The listing builds one solid part. Answer for the finished solid, in the listing's coordinates (mm). A direction names the side the tool comes from. Coordinates: 2 decimals unless noted, no trailing zeros. Order: outer loops, then holes, each group sorted by start corner. A loop starts at its lowest first (then second) coordinate and runs counter-clockwise, first axis right, second up.
```python
from build123d import *
from build123d.topology import SkipClean

# Parameters (mm, degrees)
SKETCH2_R           = 24
BOSS_EXTRUDE1_DEPTH = 47
SKETCH3_R           = 26
BOSS_EXTRUDE2_DEPTH = 14
SKETCH5_R           = 16
BOSS_EXTRUDE3_DEPTH = 46
BOSS_EXTRUDE4_START = 28
BOSS_EXTRUDE4_DEPTH = 18
SKETCH8_R           = 20
CUT_EXTRUDE1_DEPTH  = 5
SKETCH12_R          = 12.5
CUT_EXTRUDE3_DEPTH  = 34
CUT_EXTRUDE4_START  = -25
SKETCH13_R          = 12.5
CUT_EXTRUDE4_DEPTH  = 25
SKETCH11_R          = 17.5
CUT_EXTRUDE2_DEPTH  = 39
SKETCH16_W          = 29
SKETCH16_H          = 2.5
SKETCH17_W          = 2.5
SKETCH17_H          = 11.435558067


with BuildPart() as part:
    # Sketch1 → Revolve1 (revolve)
    with BuildSketch(Plane.XY):
        with BuildLine():
            Line((-29, 0), (29, 0))
            ThreePointArc((29, 0), (0, 29), (-29, 0))
        make_face()
    revolve(axis=Axis((-1000, 0, 0), (1, 0, 0)))

    # Sketch2 → Boss-Extrude1 (add)
    with BuildSketch(Plane(origin=(0, 0, 0), x_dir=(1, 0, 0), z_dir=(0, 1, 0))):
        with Locations(Location((0, 0, 0), (0, 0, 90))):
            Circle(SKETCH2_R)
    extrude(amount=BOSS_EXTRUDE1_DEPTH)

    # Sketch3 → Boss-Extrude2 (add)
    with BuildSketch(Plane(origin=(0, 47, 0), x_dir=(1, 0, 0), z_dir=(0, 1, 0))):
        with Locations(Location((0, 0, 0), (0, 0, 270))):
            Circle(SKETCH3_R)
    extrude(amount=-BOSS_EXTRUDE2_DEPTH)

    # Sketch5 → Boss-Extrude3 (add)
    with BuildSketch(Plane.XY):
        with Locations(Location((0, 0, 0), (0, 0, 180))):
            Circle(SKETCH5_R)
    boss_extrude3 = extrude(amount=BOSS_EXTRUDE3_DEPTH)

    # Sketch4 → Boss-Extrude4 (add)
    with BuildSketch(Plane.XY.offset(BOSS_EXTRUDE4_START)):
        Polygon((20.784609691, 12), (0, 24), (-20.784609691, 12), (-20.784609691, -12), (0, -24), (20.784609691, -12), align=None)
    boss_extrude4 = extrude(amount=BOSS_EXTRUDE4_DEPTH)

    # Sketch8 → Cut-Extrude1 (cut)
    with BuildSketch(Plane(origin=(0, 47, 0), x_dir=(1, 0, 0), z_dir=(0, 1, 0))):
        with Locations(Location((0, 0, 0), (0, 0, 270))):
            Circle(SKETCH8_R)
    extrude(amount=-CUT_EXTRUDE1_DEPTH, mode=Mode.SUBTRACT)

    # Sketch12 → Cut-Extrude3 (cut)
    with BuildSketch(Plane.XY.offset(46)):
        Circle(SKETCH12_R)
    extrude(amount=-CUT_EXTRUDE3_DEPTH, mode=Mode.SUBTRACT)

    # Mirror1: Boss-Extrude3, Boss-Extrude4 across plane
    add(boss_extrude3.mirror(Plane.XY))
    add(boss_extrude4.mirror(Plane.XY))

    # Sketch13 → Cut-Extrude4 (cut)
    with BuildSketch(Plane(origin=(0, 0, -46), x_dir=(-1, 0, 0), z_dir=(0, 0, -1)).offset(CUT_EXTRUDE4_START)):
        with Locations(Location((0, 0, 0), (0, 0, 180))):
            Circle(SKETCH13_R)
    extrude(amount=CUT_EXTRUDE4_DEPTH, mode=Mode.SUBTRACT)

    # Sketch11 → Cut-Extrude2 (cut)
    with BuildSketch(Plane(origin=(0, 42, 0), x_dir=(1, 0, 0), z_dir=(0, 1, 0))):
        with Locations(Location((0, 0, 0), (0, 0, 270))):
            Circle(SKETCH11_R)
    extrude(amount=-CUT_EXTRUDE2_DEPTH, mode=Mode.SUBTRACT)

    # Sketch15 → Cut-Revolve1 (revolve, cut)
    with BuildSketch(Plane(origin=(0, 0, 0), x_dir=(0, 0, -1), z_dir=(1, 0, 0))):
        Polygon((-6.5, 3), (0, -3.5), (0, 11), (-6.5, 11), align=None)
    revolve(axis=Axis((0, -1000, 0), (0, 1, 0)), mode=Mode.SUBTRACT)

    # Sketch16 → Cut-Revolve2 (revolve, cut)
    with BuildSketch(Plane(origin=(0, 0, 0), x_dir=(0, 0, -1), z_dir=(1, 0, 0)), mode=Mode.PRIVATE) as cut_revolve2_sk:
        with Locations((12, -6.25)):
            Rectangle(SKETCH16_W, SKETCH16_H)
    revolve(cut_revolve2_sk.sketch.rotate(Axis((0, -5, 4.897022233), (0, 0, -1)), 270), axis=Axis((0, -5, 4.897022233), (0, 0, -1)), mode=Mode.SUBTRACT)

    # Sketch17 → Cut-Revolve3 (revolve, cut)
    with SkipClean():  # the faces are left unmerged after this step: merging them gives an invalid solid
        with BuildSketch(Plane(origin=(0, 0, 0), x_dir=(0, 0, -1), z_dir=(1, 0, 0))):
            with Locations((-1.25, 0.717779034)):
                Rectangle(SKETCH17_W, SKETCH17_H)
        revolve(axis=Axis((0, -5, 0), (0, 1, 0)), mode=Mode.SUBTRACT)


solid = part.part
```
(1) The mould has two halves that part along X. Classify faces 1 (the face through (20.785, 0, -37)), 2 (the face through (-1.6, 16.1, 28)), 3 (the face through (-1.639, -0.806, -2.138)): released by +X, released by -X, zero draft, split by the parting line, or undercut.
(2) Find section B-B (y = 10). Write down the section's boundary in (x, z).
(3) Find section C-C (z = -15). Write down the section's boundary in (x, y) (3 decimals).
(4) Each of these flat-tipped pins is pushed along its axis until it touches: pin 1 Ø20 at (y, z) = (4, 36) entering from -X; pin 2 Ø12.5 at (x, y) = (-0.5, 1.5) entering from +Z; pin 3 Ø12 at (y, z) = (-5, 5.5) entering from +X. Where does it stop, or does it pass through?
(5) Consider line 1 (X direction, y = 21, z = 0); line 2 (Y direction, x = 0, z = -27); line 3 (Z direction, x = 17.5, y = 1). Determine where each line is inside the solid, lowest interval first.
(6) Find section D-D (z = 22). Write down the section's boundary in (x, y).
(7) Find section A-A (z = -36.5). Write down the section's boundary in (x, y), and give its area (3 significant figures).
(8) For faces 4 (the face through (-20.785, 0, -37)), 5 (the face through (3.47, 15.62, 26.07)), 6 (the face through (5.77, -11.09, 29.24)), 7 (the face through (0.751, -2.083, 2.385)), determine the directions among +Z, -Z, +X, -X, +Y, -Y from which every point of the face is accessible in a straight line to the end or side of a thin tool.
Findings below:
1. face 1: released by +X
1. face 2: zero draft
1. face 3: undercut
2. outline: (-20.78, -46) - (-7.5, -46) - (-7.5, -21) - (7.5, -21) - (7.5, -46) - (20.78, -46) - (20.78, -28) - (12.49, -28) - (12.49, -24.19) arc R27.22 ccw to (12.49, 24.19) - (12.49, 28) - (20.78, 28) - (20.78, 46) - (7.5, 46) - (7.5, 15.81) arc R17.5 cw (long way) to (-7.5, 15.81) - (-7.5, 46) - (-20.78, 46) - (-20.78, 28) - (-12.49, 28) - (-12.49, 24.19) arc R27.22 ccw to (-12.49, -24.19) - (-12.49, -28) - (-20.78, -28) - close
3. outline: (-21.237, 33) - (-18.735, 33) - (-18.735, 16.279) arc R24.819 ccw (long way) to (18.735, 16.279) - (18.735, 33) - (21.237, 33) - (21.237, 47) - (13.229, 47) - (13.229, 42) - (9.014, 42) - (9.014, 3) - (-9.014, 3) - (-9.014, 42) - (-13.229, 42) - (-13.229, 47) - (-21.237, 47) - close; hole circle Ø5 at (0, -5)
4. pin 1: stops at x = -20.78
4. pin 2: stops at z = 12
4. pin 3: stops at x = 28.96
5. line 1: x = -24 to -17.5, 17.5 to 24
5. line 2: y = -16 to -12.5, 12.5 to 16
5. line 3: z = -46 to -28, -23.1 to 23.1, 28 to 46
6. outline: (-13.86, 33) - (-9.59, 33) - (-9.59, 16.28) arc R18.89 ccw (long way) to (9.59, 16.28) - (9.59, 33) - (13.86, 33) - (13.86, 47) - (-13.86, 47) - close; hole circle Ø25 at (0, 0)
7. outline: (-20.78, -12) - (0, -24) - (20.78, -12) - (20.78, 12) - (0, 24) - (-20.78, 12) - close; hole circle Ø25 at (0, 0)
7. area: 1,010 mm2
8. face 4: -Z, -X, +Y, -Y
8. face 5: none
8. face 6: +Z
8. face 7: +Y
